Here's the drawing with two shaded views (mm, measured from the low corner). I have some questions. Coordinates: 2 decimals unless noted, no trailing zeros. Order: outer loops, then holes, each group sorted by start corner. A loop starts at its lowest first (then second) coordinate and runs counter-clockwise, first axis right, second up. Notation, with made-up numbers: (-11, -9.5) -> (33, -9.5) arc R24 cw to (33, 0.5) -> close; hole circle Ø5 at (-1.75, 21). An arc over 180 degrees is marked (long way). Answer in a Markdown table with one row per item. Add a question column.
1. Imagine slicing it at B-B on z = 2.5. Write out the boundary of the cut face in (x, y) (1 decimal).
2. Imagine slicing it at A-A on y = 107. Write out the boundary of the cut face in (x, z).
3. Imagine slicing it at C-C on x = 115. Write out the boundary of the cut face in (y, z), plus the area to 3 significant figures.
4. If I drill on line 1 along Y through (x, z) = (28, 4.5); line 2 along X through (y, z) = (31, 8.75); line 3 along Y through (x, z) = (90, 3.5), over which ranges is the centre line in solid material (lowest first)? Write a range as [from, to].
5. Will these pins go through, and if not, where does the flat tip stop? pin 1 (6 mm diameter, centred on x = 147.5, z = 4, fed in from +Y); pin 2 (1.5 mm diameter, centred on x = 94.5, z = 9.5, fed in from +Y); pin 3 (6 mm diameter, centred on y = 164.5, z = 7.5, fed in from +X).
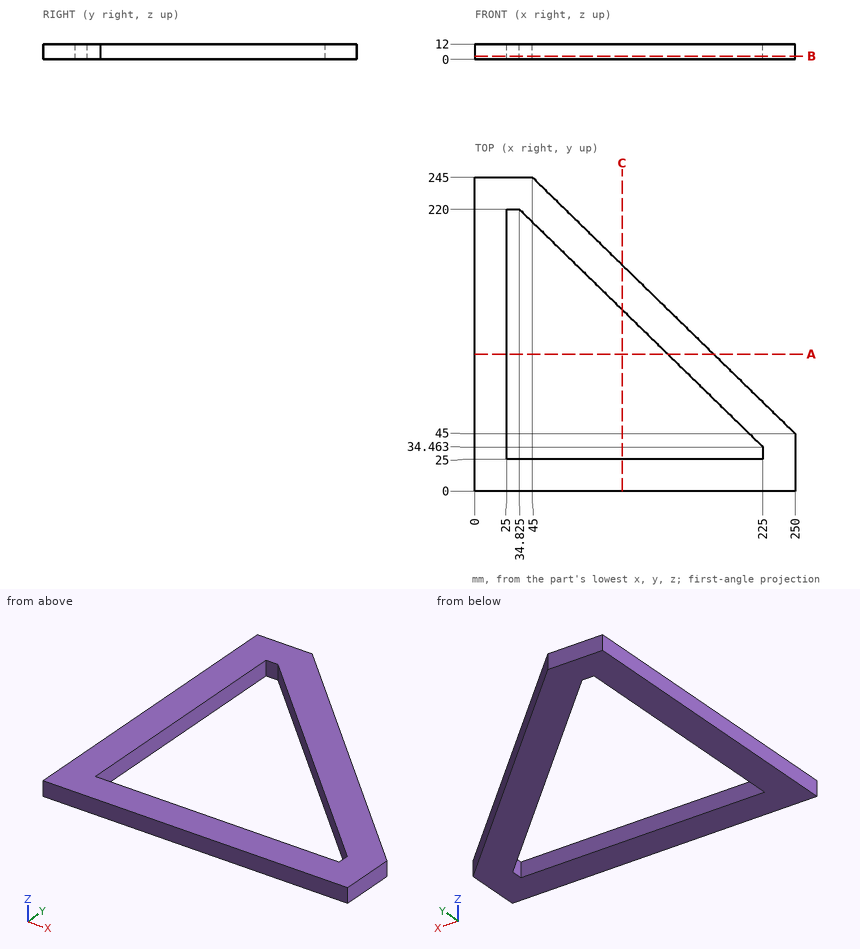
Answers follow:
| question | item | result |
|---|---|---|
| 1 | outline | (0, 0) -> (250, 0) -> (250, 45) -> (45, 245) -> (0, 245) -> close; hole (25, 25) -> (225, 25) -> (225, 34.5) -> (34.8, 220) -> (25, 220) -> close |
| 2 | outline | (0, 0) -> (25, 0) -> (25, 12) -> (0, 12) -> close; (150.65, 0) -> (186.45, 0) -> (186.45, 12) -> (150.65, 12) -> close |
| 3 | outline | (0, 0) -> (25, 0) -> (25, 12) -> (0, 12) -> close; (141.78, 0) -> (176.71, 0) -> (176.71, 12) -> (141.78, 12) -> close |
| 3 | area | 719 mm² |
| 4 | line 1 | y = [0, 25], [220, 245] |
| 4 | line 2 | x = [0, 25], [225, 250] |
| 4 | line 3 | y = [0, 25], [166.17, 201.1] |
| 5 | pin 1 | stops at y = 147.93 |
| 5 | pin 2 | stops at y = 197.44 |
| 5 | pin 3 | stops at x = 130.59 |
